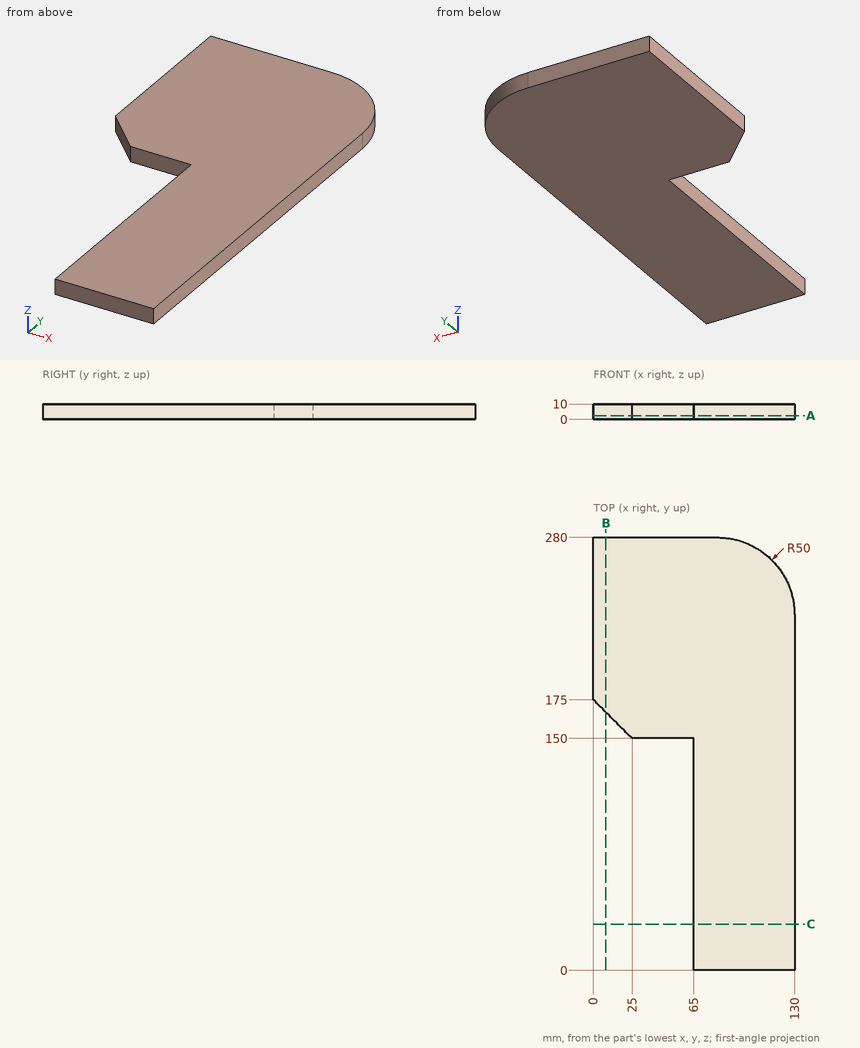
Input: dimensioned drawing with shaded views. Units: mm. Origin: part minimum x, y, z. Coordinates: 2 decimals unless noted, no trailing zeros. Write each loop counter-clockwise with the first axis right and the second up, starting at its lowest first coordinate (ties: lowest second). Pieces come first, ordered by that corner, then holes. Notation, with made-up numbers: M 66,36 L 103,36 A24 cw 103,67 Z; hole C 7.25,-2.75 d8. An arc over 180 degrees is marked long. Use one line per item in the form item = value.
Q1. First-contact query: pin 1 (1.5 mm diameter, centred on y = 31, z = 4.5, fed in from -X). Flat tip, straight axial feed; report the tip coordinate or a pass-through.
Answer below:
pin_1 = 65
Q2. Section A-A (z = 2.5). Return loops of the section in (x, y).
Answer below:
outline = M 0,175 L 25,150 L 65,150 L 65,0 L 130,0 L 130,230 A50 ccw 80,280 L 0,280 Z
Q3. Material intervals for probe 1 along X at (y, z) = (127.5, 9); probe 2 along Y at (x, z) = (40.5, 1.25); probe 3 along Y at (x, z) = (80.5, 3), sorted ascending. Write a range as from..to.
Answer below:
probe_1 = 65..130
probe_2 = 150..280
probe_3 = 0..280
Q4. Section C-C (y = 30). Return loops of the section in (x, z), plus the area to 3 significant figures.
Answer below:
outline = M 65,0 L 130,0 L 130,10 L 65,10 Z
area = 650 mm²
Q5. Section B-B (x = 8). Return loops of the section in (y, z).
Answer below:
outline = M 167,0 L 280,0 L 280,10 L 167,10 Z
